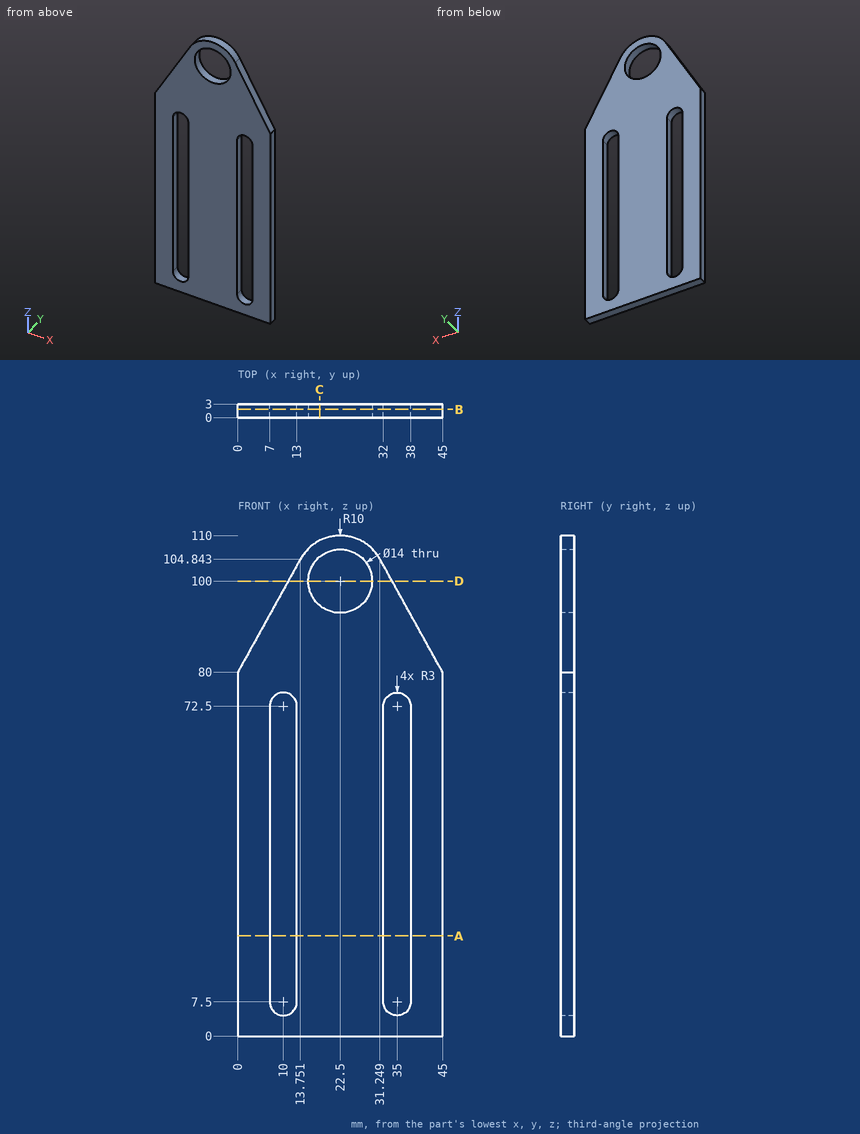
Drawing for the job (mm, zero at the part's lowest x, y, z). Give positions to 0.01 mm unless a question says otherwise; leave off trailing zeros. Write each loop counter-clockwise with the first axis right and the second up, starting at its lowest first coordinate (ties: lowest second). Pieces come first, ordered by that corner, then holes. Notation, with made-up numbers: (22, 0) -> (49, 0) arc R20 cw to (49, 33) -> close; hole circle Ø8 at (-11, -15). An arc over 180 degrees is marked (long way). Put each result on its own line as item: value. Start each with the question number.
Item 1: Pin check, flat tip, straight feed: pin 1 Ø1.5 at (y, z) = (0.5, 95) entering from -X. Stop position of the tip, or through.
Item 2: Cut at D-D (z = 100). List the corners of the cut face in (x, y), then the cut area to 3 significant figures.
Item 3: Cut at A-A (z = 22). List the corners of the cut face in (x, y).
Item 4: Cut at C-C (x = 18). List the corners of the cut face in (y, z), then the cut area to 3 significant figures.
Item 5: Wall check: L1, parallel to X at y = 2.95, z = 47.5; L2, parallel to Z at x = 7.5, y = 2.3; L3, parallel to X at y = 1, z = 5.5 (1 decimal). Give the ranges that are in metal, low to high. Write a range as [from, to].
Item 6: Cut at B-B (y = 1.8). List the corners of the cut face in (x, z), then the cut area to 3 significant figures.
Answer list:
1. pin 1: stops at x = 7.89
2. outline: (11.07, 0) -> (15.5, 0) -> (15.5, 3) -> (11.07, 3) -> close; (29.5, 0) -> (33.93, 0) -> (33.93, 3) -> (29.5, 3) -> close
2. area: 26.6 mm2
3. outline: (0, 0) -> (7, 0) -> (7, 3) -> (0, 3) -> close; (13, 0) -> (32, 0) -> (32, 3) -> (13, 3) -> close; (38, 0) -> (45, 0) -> (45, 3) -> (38, 3) -> close
4. outline: (0, 0) -> (3, 0) -> (3, 94.64) -> (0, 94.64) -> close; (0, 105.36) -> (3, 105.36) -> (3, 108.93) -> (0, 108.93) -> close
4. area: 295 mm2
5. L1: x = [0, 7], [13, 32], [38, 45]
5. L2: z = [0, 5.84], [74.16, 93.55]
5. L3: x = [0, 7.8], [12.2, 32.8], [37.2, 45]
6. outline: (0, 0) -> (45, 0) -> (45, 80) -> (31.25, 104.84) arc R10 ccw to (13.75, 104.84) -> (0, 80) -> close; hole (7, 7.5) arc R3 ccw to (13, 7.5) -> (13, 72.5) arc R3 ccw to (7, 72.5) -> close; hole circle Ø14 at (22.5, 100); hole (32, 7.5) arc R3 ccw to (38, 7.5) -> (38, 72.5) arc R3 ccw to (32, 72.5) -> close
6. area: 3,450 mm2
